Could you check a few things on this drawing? It's one solid part, dimensions in mm from its lowest x, y, z. Coordinates: 2 decimals unless noted, no trailing zeros. Write each loop counter-clockwise with the first axis right and the second up, starting at its lowest first coordinate (ties: lowest second). Pieces come first, ordered by that corner, then holes. Notation, with made-up numbers: (59, 30) - (68, 30) arc R32 ccw to (68, 66) - close; hole circle Ø7 at (-36.75, 20). An arc over 180 degrees is marked (long way). Answer as a JSON object with one key per item and string values. Group by question number.
1) If we section it at C-C (z = 5.5): Write out the boundary of the cut face in (x, y).
2) Will these pins go through, and if not, where does the flat tip stop? pin 1 Ø1.5 at (x, z) = (38, 8) entering from +Y; pin 2 Ø1.5 at (x, z) = (62, 3) entering from +Y; pin 3 Ø1.5 at (x, z) = (48.5, 7.5) entering from -Y.
3) If we section it at B-B (y = 35): Write out the boundary of the cut face in (x, z), plus the area to 3 significant figures.
4) If we section it at A-A (x = 35): Write out the boundary of the cut face in (y, z), plus the area to 3 significant figures.
5) Please list where these lines run through material, in increasing order: line 1 along Y through (x, z) = (35, 6); line 2 along Y through (x, z) = (62.5, 8); line 3 along X through (y, z) = (13, 4.25).
6) We'd pull the mould along X, two halves only. Please class the marked faces 1, 2 and 3: released by +X, released by -X, zero draft, split by the parting line, or undercut.
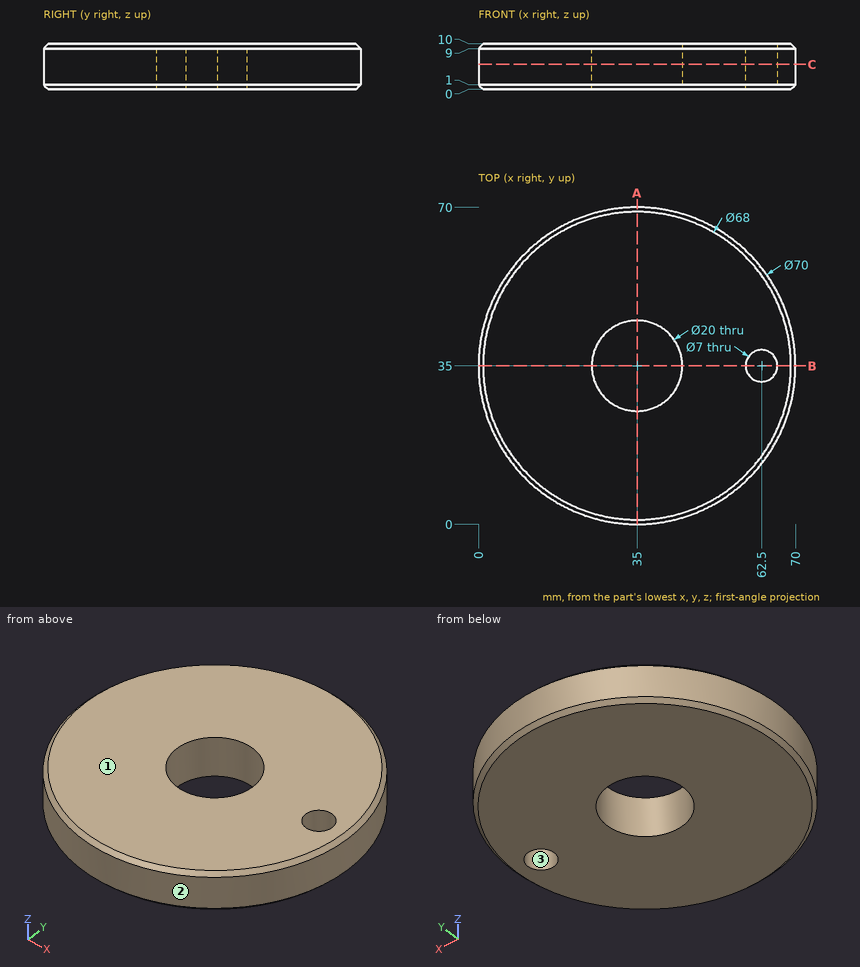
Here are the results:
{
 "1": {"outline": "circle Ø70 at (35, 35); hole circle Ø20 at (35, 35); hole circle Ø7 at (62.5, 35)"},
 "2": {"pin 1": "stops at y = 69.93", "pin 2": "stops at y = 58.15", "pin 3": "stops at y = 2.4"},
 "3": {"outline": "(0, 1) - (1, 0) - (25, 0) - (25, 10) - (1, 10) - (0, 9) - close; (45, 0) - (59, 0) - (59, 10) - (45, 10) - close; (66, 0) - (69, 0) - (70, 1) - (70, 9) - (69, 10) - (66, 10) - close", "area": "428 mm²"},
 "4": {"outline": "(0, 1) - (1, 0) - (25, 0) - (25, 10) - (1, 10) - (0, 9) - close; (45, 0) - (69, 0) - (70, 1) - (70, 9) - (69, 10) - (45, 10) - close", "area": "498 mm²"},
 "5": {"line 1": "y = 0 to 25, 45 to 70", "line 2": "y = 13.35 to 31.5, 38.5 to 56.65", "line 3": "x = 7.78 to 62.22"},
 "6": {"face 1": "zero draft", "face 2": "split by the parting line", "face 3": "undercut"}
}
